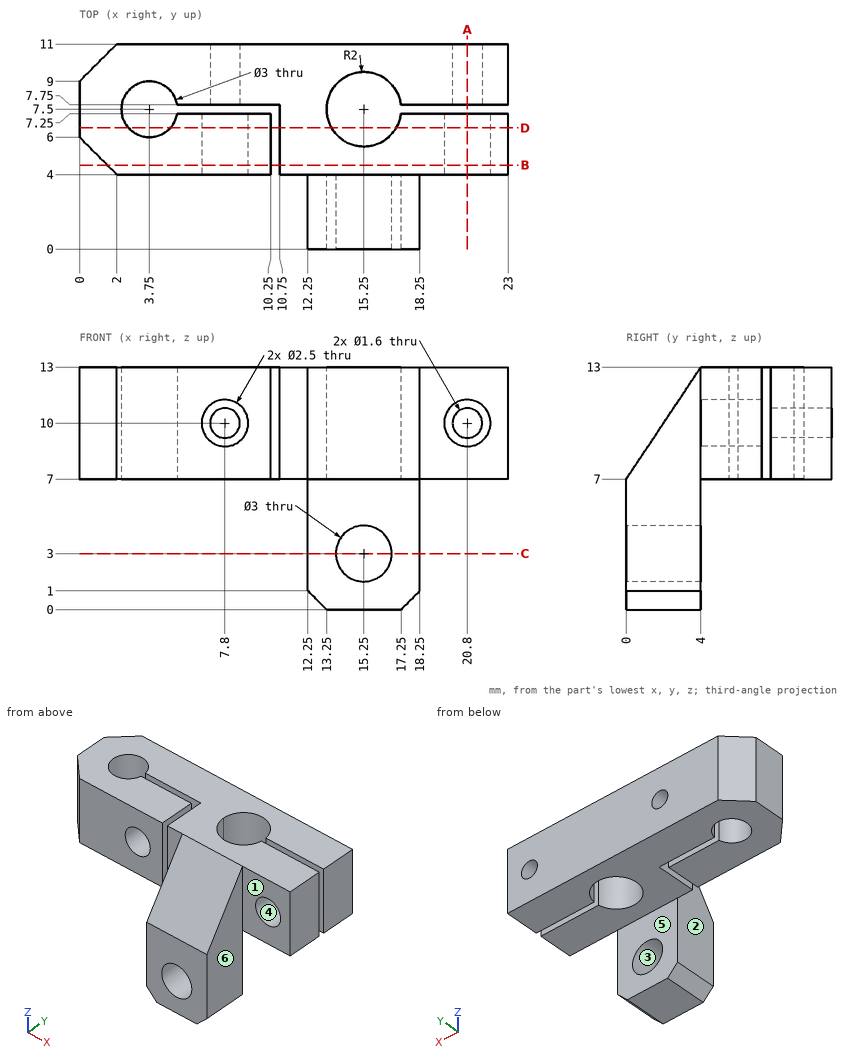
Drawing for the job (mm, zero at the part's lowest x, y, z). A direction names the side the tool comes from. Coordinates: 2 decimals unless noted, no trailing zeros. Order: outer loops, then holes, each group sorted by start corner. A loop starts at its lowest first (then second) coordinate and runs counter-clockwise, first axis right, second up. Notation, with made-up numbers: (-35, 89) -> (24, 89) arc R23 ccw to (24, 103) -> close; hole circle Ø11 at (11, 5). An arc over 180 degrees is marked (long way). Answer in a Markdown table with one row per item.
1) Mould opens along X. For the marked faces 1, 2 and 3 say: pulls with the +X half, pulls with the -X half, needs draft (parallel to the pull), parting line crosses it, or undercut.
Check values:
| item | result |
|---|---|
| face 1 | needs draft |
| face 2 | pulls with the -X half |
| face 3 | undercut |
2) Band-saw the part on D-D (y = 6.5). List the corners of the cut face in (x, z), and give its area (3 significant figures).
Check values:
| item | result |
|---|---|
| outline | (0, 7) -> (2.63, 7) -> (2.63, 13) -> (0, 13) -> close; (4.87, 7) -> (10.25, 7) -> (10.25, 13) -> (4.87, 13) -> close; (10.75, 7) -> (13.52, 7) -> (13.52, 13) -> (10.75, 13) -> close; (16.98, 7) -> (23, 7) -> (23, 13) -> (16.98, 13) -> close; hole circle Ø2.5 at (7.8, 10); hole circle Ø2.5 at (20.8, 10) |
| area | 91.0 mm2 |
3) Band-saw the part on C-C (z = 3). List the corners of the cut face in (x, y).
Check values:
| item | result |
|---|---|
| outline | (12.25, 0) -> (13.75, 0) -> (13.75, 4) -> (12.25, 4) -> close; (16.75, 0) -> (18.25, 0) -> (18.25, 4) -> (16.75, 4) -> close |
4) Band-saw the part on A-A (x = 20.8). List the corners of the cut face in (y, z).
Check values:
| item | result |
|---|---|
| outline | (4, 7) -> (7.25, 7) -> (7.25, 8.75) -> (4, 8.75) -> close; (4, 11.25) -> (7.25, 11.25) -> (7.25, 13) -> (4, 13) -> close; (7.75, 7) -> (11, 7) -> (11, 9.2) -> (7.75, 9.2) -> close; (7.75, 10.8) -> (11, 10.8) -> (11, 13) -> (7.75, 13) -> close |
5) Band-saw the part on B-B (y = 4.5). List the corners of the cut face in (x, z), and give its area (3 significant figures).
Check values:
| item | result |
|---|---|
| outline | (1.5, 7) -> (10.25, 7) -> (10.25, 13) -> (1.5, 13) -> close; (10.75, 7) -> (23, 7) -> (23, 13) -> (10.75, 13) -> close; hole circle Ø2.5 at (7.8, 10); hole circle Ø2.5 at (20.8, 10) |
| area | 116 mm2 |
6) Which spindle directions (+Z, -Z, +X, -X, +Y, -Y) get a long thin tool onto all of the face, cutting with end or side? Do the marked faces 4, 5 and 6. Say none if no direction does.
Check values:
| item | result |
|---|---|
| face 4 | -Y |
| face 5 | -Z, +X, -X, +Y |
| face 6 | +Z, -Z, +X, -Y |
7) Flat gauge pins, fed straight in: P1, Ø2.5, axis at x = 20, z = 10.5, coming from the -Y side; P2, Ø1.8, axis at x = 15.5, z = 4, coming from the +Y side; P3, Ø0.8, axis at x = 12, z = 9, coming from the -Y side. Where does each tip first touch, or does it go through?
Check values:
| item | result |
|---|---|
| P1 | y = 4 |
| P2 | y = 4 |
| P3 | y = 1.13 |
8) Drill centre lines: line 1 (Z direction, x = 7.8, y = 4.9); line 2 (Y direction, x = 7, z = 9); line 3 (Y direction, x = 3.75, z = 10.35). Where is each one in solid material? Low to high.
Check values:
| item | result |
|---|---|
| line 1 | 7 to 8.75, 11.25 to 13 |
| line 2 | 4 to 7.25, 7.75 to 11 |
| line 3 | 4 to 6, 9 to 11 |
